Verification items for the finished model (mm, model axes). A direction names the side the tool comes from. Coordinates: 2 decimals unless noted, no trailing zeros. Order: outer loops, then holes, each group sorted by start corner. A loop starts at its lowest first (then second) coordinate and runs counter-clockwise, first axis right, second up. Notation, with made-up numbers: M 36.25,2.25 L 40.25,2.25 A23 ccw 40.25,20.25 Z; hole C 71,53.25 d2. An arc over 180 degrees is marked long. Write item = value, one per line.
```python
from build123d import *

# Parameters (mm, degrees)
BASE_PLATE_SKETCH_W     = 68
BASE_PLATE_SKETCH_H     = 70
BASE_PLATE_16MM_DEPTH   = 16
C_SIDE_FLANGE_8MM_DEPTH = 8
WINDOW_CUT_OUT_DEPTH    = 18


with BuildPart() as part:
    # Base Plate Sketch → Base Plate 16mm (new body)
    with BuildSketch(Plane.XY):
        with Locations((34, 35)):
            Rectangle(BASE_PLATE_SKETCH_W, BASE_PLATE_SKETCH_H)
    extrude(amount=BASE_PLATE_16MM_DEPTH)

    # Side Flange Sketch → C Side Flange 8mm (add)
    with BuildSketch(Plane.ZY):
        Polygon((16, 70), (56, 70), (56, 58), (30, 58), (30, 12), (56, 12), (56, 0), (16, 0), (0, 0), (0, 70), align=None)
    extrude(amount=-C_SIDE_FLANGE_8MM_DEPTH)

    # Window Sketch → Window Cut-Out (cut)
    with BuildSketch(Plane.XY.offset(16)):
        Polygon((58, 18), (18, 18), (29, 52), (38, 52), (47, 52), align=None)
    extrude(amount=-WINDOW_CUT_OUT_DEPTH, mode=Mode.SUBTRACT)


solid = part.part
```
Item 1: Sectioned sample at A-A, the plane z = 13. Enter the section's corners in (x, y), then the cut area to 3 significant figures.
Report:
outline = M 0,0 L 68,0 L 68,70 L 0,70 Z; hole M 18,18 L 58,18 L 47,52 L 29,52 Z
area = 3,770 mm^2
Item 2: Scan lines: L1, parallel to Y at x = 3, z = 33.5; L2, parallel to Z at x = 58, y = 39; L3, parallel to X at y = 22, z = 21. Record each from-to range of solid material in increasing order. Write a range as from..to.
Report:
L1 = 0..12, 58..70
L2 = 0..16
L3 = 0..8
Item 3: Release check for a two-part mould opening along X. For faces 1 (the flat face through (0, 35, 22)), 2 (the flat face through (26, 0, 15)), 3 (the flat face through (23.423, 34.762, 8.112)) record: pulls with the +X half, pulls with the -X half, needs draft (parallel to the pull), parting line crosses it, or undercut.
Report:
face_1 = pulls with the -X half
face_2 = needs draft
face_3 = undercut
Item 4: Tool access check on faces 4 (the flat face through (68, 35, 8)), 5 (the flat face through (38, 18, 8)), 6 (the flat face through (4, 12, 43)), 7 (the flat face through (8, 35, 27)). Record the directions out of +Z, -Z, +X, -X, +Y, -Y that give a thin tool (end or side, any length) a straight path to the whole face; none if there is none.
Report:
face_4 = +Z, -Z, +X, +Y, -Y
face_5 = +Z, -Z
face_6 = +Z, +X, -X
face_7 = +Z, +X, +Y, -Y
Item 5: Sectioned sample at D-D, the plane y = 46. Enter the section's corners in (x, z).
Report:
outline = M 0,0 L 27.06,0 L 27.06,16 L 8,16 L 8,30 L 0,30 Z; M 48.94,0 L 68,0 L 68,16 L 48.94,16 Z
Item 6: Sectioned sample at B-B, the plane x = 39. Enter the section's corners in (y, z).
Report:
outline = M 0,0 L 18,0 L 18,16 L 0,16 Z; M 52,0 L 70,0 L 70,16 L 52,16 Z
Item 7: Sectioned sample at C-C, the plane z = 51. Enter the section's corners in (x, y), then the cut area to 3 significant figures.
Report:
outline = M 0,0 L 8,0 L 8,12 L 0,12 Z; M 0,58 L 8,58 L 8,70 L 0,70 Z
area = 192 mm^2
Item 8: Gauge pin test, flat ends, axial feed: pin 1 (12 mm diameter, centred on y = 28, z = 30.5, fed in from +X); pin 2 (8 mm diameter, centred on x = 40.5, y = 19.5, fed in from +Z); pin 3 (6.5 mm diameter, centred on x = 6, y = 27, fed in from +Z). Record the tip position at first contact, or that the pin passes through.
Report:
pin_1 = 8
pin_2 = 16
pin_3 = 30
